Verification items for the finished model (mm, model axes). A direction names the side the tool comes from. Give positions to 0.01 mm unless a question says otherwise; leave off trailing zeros. Order: outer loops, then holes, each group sorted by start corner. A loop starts at its lowest first (then second) coordinate and runs counter-clockwise, first axis right, second up.
(1) Gauge pin test, flat ends, axial feed: pin 1 (2.5 mm diameter, centred on x = 0, y = 8, fed in from +Z); pin 2 (1.5 mm diameter, centred on y = 7.5, z = 3, fed in from -X); pin 3 (1.5 mm diameter, centred on y = 7, z = 1, fed in from +X); pin 4 (4 mm diameter, centred on x = -4, y = -9, fed in from +Z). Record the tip position at first contact, or that the pin passes through.
(2) Scan lines: L1, parallel to Y at x = 0, z = 1.75; L2, parallel to Z at x = -9.5, y = -9.5; L3, parallel to X at y = 2.25, z = 2.5. Record each from-to range of solid material in increasing order.
(3) Sectioned sample at B-B on y = 0. Record the cut outline in (x, z).
(4) Sectioned sample at A-A on x = 0. Record the cut outline in (y, z), plus the area to 3 significant figures.
(5) Mould release check, pull along Y, two halves, no side actions. Record for faces 1 (the face through (0, 10, 3)), 2 (the face through (1, 6, 6)), 3 (the face through (0, 12, 3)): pulls with the +Y half, pulls with the -Y half, needs draft (parallel to the pull), parting line crosses it, or undercut.
(6) Sectioned sample at D-D on x = 3. Record the cut outline in (y, z), plus the area to 3 significant figures.
(7) Access from +Z, -Z, +X, -X, +Y, -Y to the whole of each face (thin tool, end or side, straight path). Record for faces 4 (the face through (0, -8, 6)), 5 (the face through (-0.867, -3.905, 3.204)).
(8) Sectioned sample at C-C on z = 5.5. Record the cut outline in (x, y).
```python
from build123d import *

# Parameters (mm, degrees)
SKETCH1_R           = 4
BOSS_EXTRUDE2_DEPTH = 6
SKETCH3_R           = 2
BOSS_EXTRUDE3_DEPTH = 6
SKETCH4_R           = 5.5
SKETCH4_R_2         = 4
BOSS_EXTRUDE4_DEPTH = 0.5


with BuildPart() as part:
    # Sketch1 → Boss-Extrude2 (new body)
    with BuildSketch(Plane.XY):
        with BuildLine():
            Line((-5.300838508, -1.466666667), (-14.456832295, -4))
            ThreePointArc((-14.456832295, -4), (0, -15), (14.456832295, -4))
            Line((14.456832295, -4), (5.300838508, -1.466666667))
            ThreePointArc((5.300838508, -1.466666667), (0, 5.5), (-5.300838508, -1.466666667))
        make_face()
        Circle(SKETCH1_R, mode=Mode.SUBTRACT)
    extrude(amount=BOSS_EXTRUDE2_DEPTH)

    # Sketch3 → Boss-Extrude3 (add)
    with BuildSketch(Plane.XY):
        with BuildLine():
            Line((-3.929058411, 8.75), (-5.402455316, 1.03125))
            ThreePointArc((-5.402455316, 1.03125), (0, 5.5), (5.402455316, 1.03125))
            Line((5.402455316, 1.03125), (3.929058411, 8.75))
            ThreePointArc((3.929058411, 8.75), (0, 12), (-3.929058411, 8.75))
        make_face()
        with Locations((0, 8)):
            Circle(SKETCH3_R, mode=Mode.SUBTRACT)
    extrude(amount=BOSS_EXTRUDE3_DEPTH)

    # Sketch4 → Boss-Extrude4 (add)
    with BuildSketch(Plane.XY.offset(6)):
        with Locations(Location((0, 0, 0), (0, 0, 169.193077125))):
            Circle(SKETCH4_R)
        Circle(SKETCH4_R_2, mode=Mode.SUBTRACT)
    extrude(amount=BOSS_EXTRUDE4_DEPTH)


solid = part.part
```
Ans:
1. pin 1: passes through
1. pin 2: stops at x = -4.31
1. pin 3: stops at x = 4.41
1. pin 4: stops at z = 6
2. L1: y = -15 to -4, 4 to 6, 10 to 12
2. L2: z = 0 to 6
2. L3: x = -5.17 to -3.31, 3.31 to 5.17
3. outline: (-5.5, 0) - (-4, 0) - (-4, 6.5) - (-5.5, 6.5) - close; (4, 0) - (5.5, 0) - (5.5, 6.5) - (4, 6.5) - close
4. outline: (-15, 0) - (-4, 0) - (-4, 6.5) - (-5.5, 6.5) - (-5.5, 6) - (-15, 6) - close; (4, 0) - (6, 0) - (6, 6) - (5.5, 6) - (5.5, 6.5) - (4, 6.5) - close; (10, 0) - (12, 0) - (12, 6) - (10, 6) - close
4. area: 91.5 mm2
5. face 1: undercut
5. face 2: needs draft
5. face 3: pulls with the +Y half
6. outline: (-14.7, 0) - (-2.65, 0) - (-2.65, 6.5) - (-4.61, 6.5) - (-4.61, 6) - (-14.7, 6) - close; (2.65, 0) - (10.65, 0) - (10.65, 6) - (4.61, 6) - (4.61, 6.5) - (2.65, 6.5) - close
6. area: 122 mm2
7. face 4: +Z, -Y
7. face 5: +Z, -Z
8. outline: (-14.46, -4) arc R15 ccw to (14.46, -4) - (5.3, -1.47) arc R5.5 ccw to (5.4, 1.03) - (3.93, 8.75) arc R4 ccw to (-3.93, 8.75) - (-5.4, 1.03) arc R5.5 ccw to (-5.3, -1.47) - close; hole circle Ø8 at (0, 0); hole circle Ø4 at (0, 8)
